Work out the finished part from the listing and answer in its coordinate system (mm). Give positions to 0.01 mm unless a question says otherwise; leave off trailing zeros. Write each loop counter-clockwise with the first axis right and the second up, starting at its lowest first coordinate (ties: lowest second). Pieces come first, ordered by that corner, then holes.
1) Find section B-B (x = 872.5). Determine the outline of the cut face in (y, z), plus the area to 3 significant figures.
2) Straight lines are drawn through the part: probe 1 along X at (y, z) = (400, 2.6); probe 2 along X at (y, z) = (298, 3.1); probe 3 along Y at (x, z) = (-847.5, 1.3). For each, find the intervals that lie inside material, in ascending order.
3) Find section A-A (z = 2.7). Count the separate pieces of the cut face and the enclosed holes in it, plus the area to 3 significant figures.
4) Given pin 1 Ø1.2 at (x, z) = (1058.5, 3) entering from -Y, flat-ended and moving along its own axis, determine where the tip first touches the part or whether it passes through.
```python
from build123d import *

# Parameters (mm, degrees)
BOSS_EXTRUDE1_DEPTH = 4
SKETCH2_R           = 3.5
SKETCH2_R_2         = 4.5
CUT_EXTRUDE1_DEPTH  = 4


with BuildPart() as part:
    # Sketch1 → Boss-Extrude1 (new body)
    with BuildSketch(Plane.XY):
        Polygon((-790, 570), (-790, 413), (-992.5, 413), (-992.5, 255), (-1110, 255), (-1110, -445), (-790, -445), (-790, -570), (790, -570), (790, -445), (1110, -445), (1110, 255), (992.5, 255), (992.5, 413), (790, 413), (790, 570), align=None)
    extrude(amount=BOSS_EXTRUDE1_DEPTH)

    # Sketch2 → Cut-Extrude1 (cut)
    with BuildSketch(Plane.XY.offset(4)):
        with Locations((-760, 400)):
            Circle(SKETCH2_R)
        with Locations((-260, 400)):
            Circle(SKETCH2_R)
        with Locations((240, 400)):
            Circle(SKETCH2_R)
        with Locations((740, 400)):
            Circle(SKETCH2_R)
        with Locations((-760, -75)):
            Circle(SKETCH2_R)
        with Locations((-260, -75)):
            Circle(SKETCH2_R)
        with Locations((240, -75)):
            Circle(SKETCH2_R)
        with Locations((740, -75)):
            Circle(SKETCH2_R)
        with Locations((-760, -550)):
            Circle(SKETCH2_R)
        with Locations((-260, -550)):
            Circle(SKETCH2_R)
        with Locations((240, -550)):
            Circle(SKETCH2_R)
        with Locations((740, -550)):
            Circle(SKETCH2_R)
        with Locations((-922.5, 298)):
            Circle(SKETCH2_R_2)
        with Locations((-847.5, 298)):
            Circle(SKETCH2_R_2)
        with Locations((-922.5, -202)):
            Circle(SKETCH2_R_2)
        with Locations((-847.5, -202)):
            Circle(SKETCH2_R_2)
        with Locations((847.5, 298)):
            Circle(SKETCH2_R_2)
        with Locations((922.5, 298)):
            Circle(SKETCH2_R_2)
        with Locations((847.5, -202)):
            Circle(SKETCH2_R_2)
        with Locations((922.5, -202)):
            Circle(SKETCH2_R_2)
        with BuildLine():
            Line((-1065.5, 217.5), (-1054.5, 217.5))
            ThreePointArc((-1054.5, 217.5), (-1050, 213), (-1054.5, 208.5))
            Line((-1054.5, 208.5), (-1065.5, 208.5))
            ThreePointArc((-1065.5, 208.5), (-1070, 213), (-1065.5, 217.5))
        make_face()
        with BuildLine():
            Line((-1065.5, 17.5), (-1054.5, 17.5))
            ThreePointArc((-1054.5, 17.5), (-1050, 13), (-1054.5, 8.5))
            Line((-1054.5, 8.5), (-1065.5, 8.5))
            ThreePointArc((-1065.5, 8.5), (-1070, 13), (-1065.5, 17.5))
        make_face()
        with BuildLine():
            Line((-1065.5, -182.5), (-1054.5, -182.5))
            ThreePointArc((-1054.5, -182.5), (-1050, -187), (-1054.5, -191.5))
            Line((-1054.5, -191.5), (-1065.5, -191.5))
            ThreePointArc((-1065.5, -191.5), (-1070, -187), (-1065.5, -182.5))
        make_face()
        with BuildLine():
            Line((-1065.5, -382.5), (-1054.5, -382.5))
            ThreePointArc((-1054.5, -382.5), (-1050, -387), (-1054.5, -391.5))
            Line((-1054.5, -391.5), (-1065.5, -391.5))
            ThreePointArc((-1065.5, -391.5), (-1070, -387), (-1065.5, -382.5))
        make_face()
        with BuildLine():
            Line((1065.5, -382.5), (1054.5, -382.5))
            ThreePointArc((1054.5, -382.5), (1050, -387), (1054.5, -391.5))
            Line((1054.5, -391.5), (1065.5, -391.5))
            ThreePointArc((1065.5, -391.5), (1070, -387), (1065.5, -382.5))
        make_face()
        with BuildLine():
            Line((1065.5, -182.5), (1054.5, -182.5))
            ThreePointArc((1054.5, -182.5), (1050, -187), (1054.5, -191.5))
            Line((1054.5, -191.5), (1065.5, -191.5))
            ThreePointArc((1065.5, -191.5), (1070, -187), (1065.5, -182.5))
        make_face()
        with BuildLine():
            Line((1065.5, 17.5), (1054.5, 17.5))
            ThreePointArc((1054.5, 17.5), (1050, 13), (1054.5, 8.5))
            Line((1054.5, 8.5), (1065.5, 8.5))
            ThreePointArc((1065.5, 8.5), (1070, 13), (1065.5, 17.5))
        make_face()
        with BuildLine():
            Line((1065.5, 217.5), (1054.5, 217.5))
            ThreePointArc((1054.5, 217.5), (1050, 213), (1054.5, 208.5))
            Line((1054.5, 208.5), (1065.5, 208.5))
            ThreePointArc((1065.5, 208.5), (1070, 213), (1065.5, 217.5))
        make_face()
    extrude(amount=-CUT_EXTRUDE1_DEPTH, mode=Mode.SUBTRACT)


solid = part.part
```
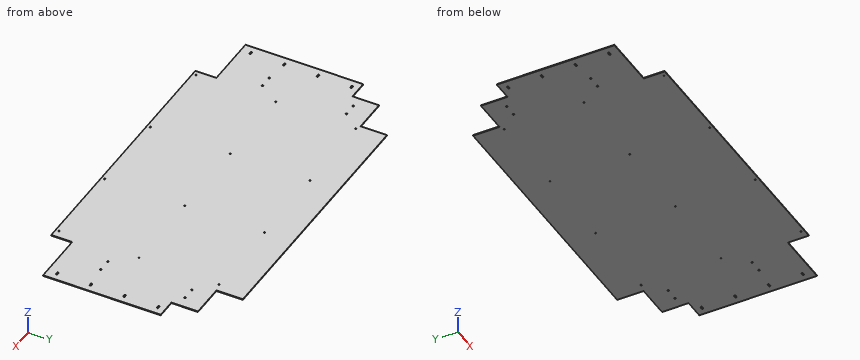
Results:
1. outline: (-445, 0) - (413, 0) - (413, 4) - (-445, 4) - close
1. area: 3,430 mm2
2. probe 1: x = -992.5 to -763.5, -756.5 to -263.5, -256.5 to 236.5, 243.5 to 736.5, 743.5 to 992.5
2. probe 2: x = -992.5 to -927, -918 to -852, -843 to 843, 852 to 918, 927 to 992.5
2. probe 3: y = -445 to -206.5, -197.5 to 293.5, 302.5 to 413
3. separate pieces: 1
3. enclosed holes: 28
3. area: 2,310,000 mm2
4. pin 1: stops at y = -445
